Can you work these out from the model? Positions are in its coordinate system, mm. A direction names the side the tool comes from. Round coordinates to 2 decimals unless told otherwise and drop trailing zeros. Write each loop counter-clockwise with the first axis right and the second up, starting at its lowest first coordinate (ties: lowest second). Pieces come first, ordered by that corner, then holes. Notation, with made-up numbers: M -35,-9 L -6,-9 A29 cw -6,18 Z; hole C 56,-17.5 d6. An arc over 180 degrees is marked long. Use one line per item in the form item = value. Start each with the question number.
```python
from build123d import *

# Parameters (mm, degrees)
FILLET1_R             = 1
CHAMFER1_SIZE         = 0.5
CHAMFER2_SIZE         = 1
M5_TAPPED_HOLE1_D     = 4.2
M5_TAPPED_HOLE1_DEPTH = 14
M5_TAPPED_HOLE1_TIP   = 1.2618073


with BuildPart() as part:
    # Sketch1 → Revolve1 (revolve)
    with BuildSketch(Plane.XY, mode=Mode.PRIVATE) as revolve1_sk:
        Polygon((13, 6.5), (13, 9), (17, 9), (17, 6.25), (18, 6.25), (18, 6.5), (93, 6.5), (93, 0), (0, 0), (0, 6.5), align=None)
    revolve(revolve1_sk.sketch.rotate(Axis((0, 0, 0), (1, 0, 0)), 90), axis=Axis((0, 0, 0), (1, 0, 0)))

    # Fillet1
    fillet1_edges = [part.edges().sort_by_distance(p)[0] for p in [
        (93, 0, -6.5),
    ]]
    fillet(fillet1_edges, radius=FILLET1_R)

    # Chamfer1
    chamfer1_edges = [part.edges().sort_by_distance(p)[0] for p in [
        (13, 0, -9),
    ]]
    chamfer(chamfer1_edges, length=CHAMFER1_SIZE)

    # Chamfer2
    chamfer2_edges = [part.edges().sort_by_distance(p)[0] for p in [
        (0, 0, -6.5),
    ]]
    chamfer(chamfer2_edges, length=CHAMFER2_SIZE)

    # M5 Tapped Hole1
    with Locations(Plane.ZY):
        with Locations((0, 0)):
            Hole(M5_TAPPED_HOLE1_D / 2, depth=M5_TAPPED_HOLE1_DEPTH)
            with Locations((0, 0, -(M5_TAPPED_HOLE1_DEPTH + M5_TAPPED_HOLE1_TIP / 2))):  # 118° drill point
                Cone(0, M5_TAPPED_HOLE1_D / 2, M5_TAPPED_HOLE1_TIP, mode=Mode.SUBTRACT)


solid = part.part
```
1. If we mould it in two halves opening along X, with no side actions, what happens to faces 1 (the face through (15.274, -6.083, -6.633)), 2 (the face through (17.51, -1.88, 5.96)), 3 (the face through (15.04, -0.14, 0.34)), 4 (the face through (93, 0, 0))? For each: pulls with the +X half, pulls with the -X half, needs draft (parallel to the pull), parting line crosses it, or undercut.
2. Will these pins go through, and if not, where does the flat tip stop? pin 1 (6 mm diameter, centred on x = 44, z = 4, fed in from -Y); pin 2 (1 mm diameter, centred on x = 71.5, y = -4.5, fed in from -Z); pin 3 (1.5 mm diameter, centred on x = 38, y = 6, fed in from +Z).
3. Which directions (+Z, -Z, +X, -X, +Y, -Y) give clear straight access to the entire face, cutting with the end or side of a thin tool? Please do faces 5 (the face through (7.084, 3.955, -5.158)), 6 (the face through (0, 2.4, 0.1)).
4. Please list where these lines run through material, in increasing order: line 1 along Y through (x, z) = (10.75, 0); line 2 along X through (y, z) = (-3.25, -6.5); line 3 along Y through (x, z) = (72, 2.75).
5. If we section it at A-A (x = 39.5): List the corners of the cut face in (y, z) for me.
Model answer:
q1.face_1 = needs draft
q1.face_2 = undercut
q1.face_3 = pulls with the -X half
q1.face_4 = pulls with the +X half
q2.pin_1 = -6.42
q2.pin_2 = -5.12
q2.pin_3 = 3.83
q3.face_5 = -X
q3.face_6 = +Z, -Z, -X, +Y, -Y
q4.line_1 = -6.5 to -2.1, 2.1 to 6.5
q4.line_2 = 13 to 17
q4.line_3 = -5.89 to 5.89
q5.outline = C 0,0 d13
